Geometry check sheet. Reference: drawing and pictorial views, mm from the part's lowest x, y, z. A direction names the side the tool comes from. Round coordinates to 2 decimals unless told otherwise and drop trailing zeros. Order: outer loops, then holes, each group sorted by start corner. A loop starts at its lowest first (then second) coordinate and runs counter-clockwise, first axis right, second up. Notation, with made-up numbers: M 30.25,28 L 60.25,28 A13 ccw 60.25,48 Z; hole C 26,13.5 d2. An arc over 180 degrees is marked long. Answer as a JSON object with one key per item and string values. Group by question number.
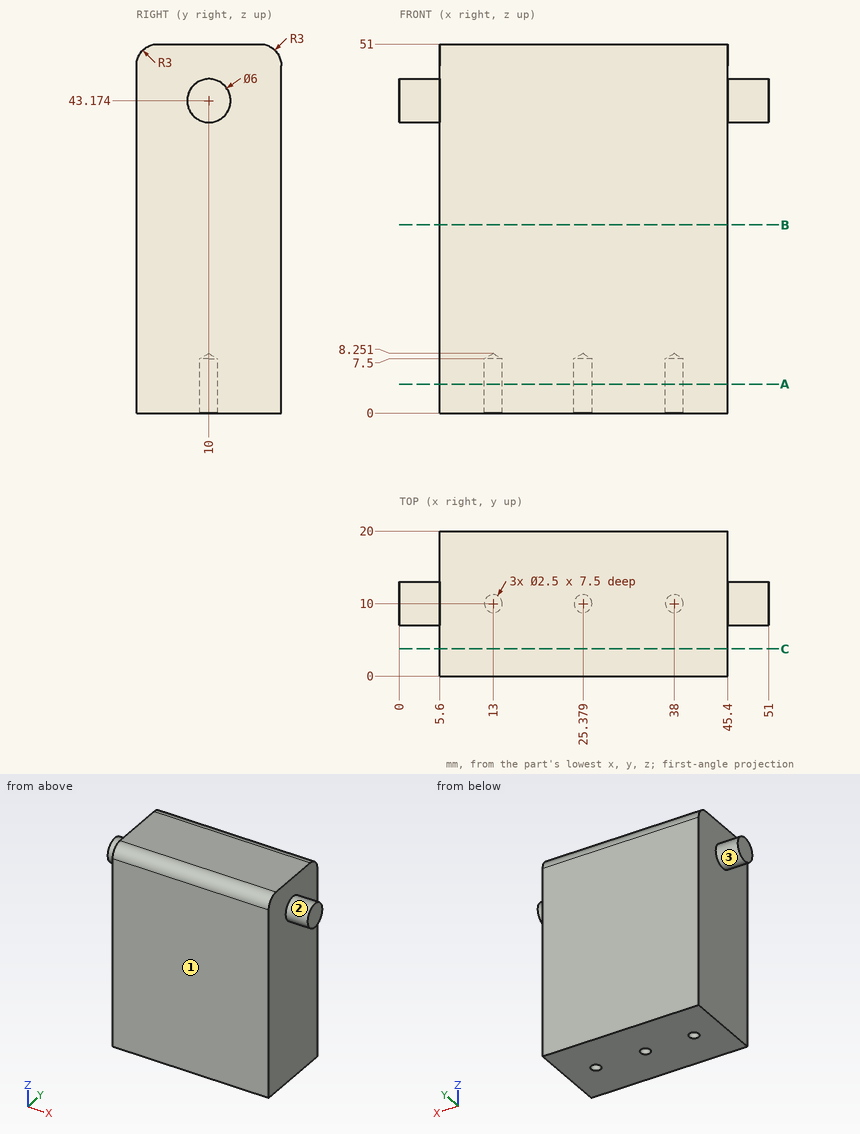
Q1. Gauge pin test, flat ends, axial feed: pin 1 Ø2 at (x, y) = (38, 10) entering from -Z; pin 2 Ø6 at (y, z) = (2, 17.5) entering from -X; pin 3 Ø5 at (y, z) = (7.5, 23) entering from +X. Record the tip position at first contact, or that the pin passes through.
Q2. Cross-section at A-A, the plane z = 4. Record the cut outline in (x, y), then the cut area to 3 significant figures.
Q3. Cross-section at B-B, the plane z = 26. Record the cut outline in (x, y), then the cut area to 3 significant figures.
Q4. Tool access check on the marked faces 1, 2 and 3. Record the directions out of +Z, -Z, +X, -X, +Y, -Y that give a thin tool (end or side, any length) a straight path to the whole face; none if there is none.
Q5. Cross-section at C-C, the plane y = 3.75. Record the cut outline in (x, z).
Q6. Thickness scan on line 1 (X direction, y = 10, z = 4.75); line 2 (Y direction, x = 13, z = 4); line 3 (X direction, y = 9.5, z = 39.5). Record the ranges inside material, lowest first. Write a range as from..to.
Conclusion:
{
 "1": {"pin 1": "z = 7.65", "pin 2": "x = 5.6", "pin 3": "x = 45.4"},
 "2": {"outline": "M 5.6,0 L 45.4,0 L 45.4,20 L 5.6,20 Z; hole C 13,10 d2.5; hole C 25.38,10 d2.5; hole C 38,10 d2.5", "area": "781 mm2"},
 "3": {"outline": "M 5.6,0 L 45.4,0 L 45.4,20 L 5.6,20 Z", "area": "796 mm2"},
 "4": {"face 1": "+Z, -Z, +X, -X, -Y", "face 2": "+X", "face 3": "-X"},
 "5": {"outline": "M 5.6,0 L 45.4,0 L 45.4,51 L 5.6,51 Z"},
 "6": {"line 1": "5.6..11.75, 14.25..24.13, 26.63..36.75, 39.25..45.4", "line 2": "0..8.75, 11.25..20", "line 3": "5.6..45.4"}
}
